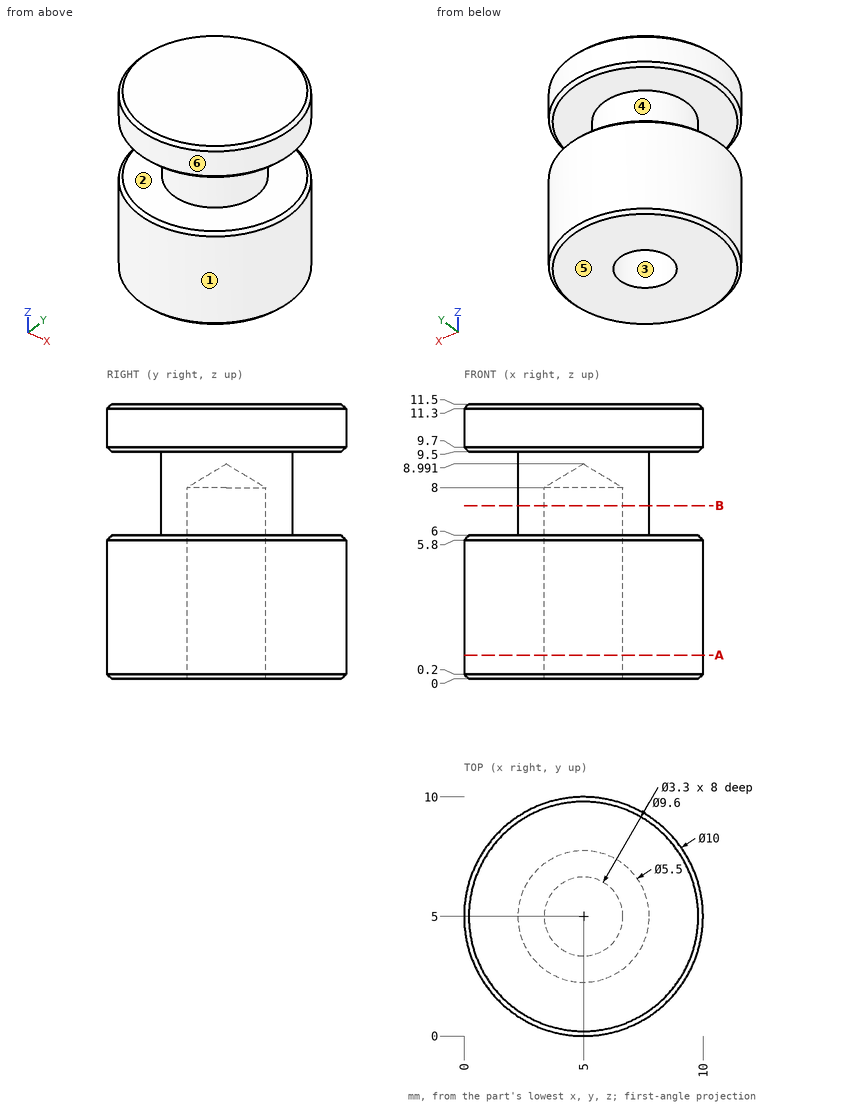
Design review of the part shown in the three views and the two pictorial views. Dimensions are in mm from the part's minimum x, y and z. A direction names the side the tool comes from. Coordinates: 2 decimals unless noted, no trailing zeros. Order: outer loops, then holes, each group sorted by start corner. A loop starts at its lowest first (then second) coordinate and runs counter-clockwise, first axis right, second up. Notation, with made-up numbers: (29, -35) - (50, -35) arc R25 cw to (50, -23) - close; hole circle Ø8 at (26.5, 21). An arc over 180 degrees is marked (long way). One line per question, with ' | ' between items.
Q1. Consider section A-A, the plane z = 1. Give the boundary of the cut face in (x, y), then the cut area to 3 significant figures.
Answer key:
outline: circle Ø10 at (5, 5); hole circle Ø3.3 at (5, 5) | area: 70.0 mm2
Q2. The part is to be moulded in two halves that separate along Z. For the marked faces 4, 5 and 6, say which applies: +Z half, -Z half, draft (parallel to the pull), parting line (faces both ways), or undercut.
Answer key:
face 4: undercut | face 5: -Z half | face 6: draft
Q3. Clearance check with flat-ended pins moving along their axes: pin 1 Ø1.5 at (x, z) = (8.5, 1.5) entering from -Y (1 decimal); pin 2 Ø2 at (x, z) = (5.5, 8) entering from -Y; pin 3 Ø2 at (x, z) = (7, 1.5) entering from +Y. State where each tip first meets the part, or that it passes through.
Answer key:
pin 1: stops at y = 0.8 | pin 2: stops at y = 2.25 | pin 3: stops at y = 9.9
Q4. Consider section B-B, the plane z = 7.25. Give the boundary of the cut face in (x, y).
Answer key:
outline: circle Ø5.5 at (5, 5); hole circle Ø3.3 at (5, 5)
Q5. To check wall thickness, follow line 1 along Y through (x, z) = (5, 5.25); line 2 along Z through (x, y) = (6, 8.75); line 3 along Y through (x, z) = (5, 6.5). State the ranges of each line that lie inside material, in increasing order.
Answer key:
line 1: y = 0 to 3.35, 6.65 to 10 | line 2: z = 0 to 6, 9.5 to 11.5 | line 3: y = 2.25 to 3.35, 6.65 to 7.75
Q6. For the marked faces 1, 2 and 3, list the 3-axis set-ups (+Z, -Z, +X, -X, +Y, -Y) from which the entire face can be reached by the end or side of a thin tool; tool diameter is ignored.
Answer key:
face 1: +Z, -Z | face 2: none | face 3: -Z
